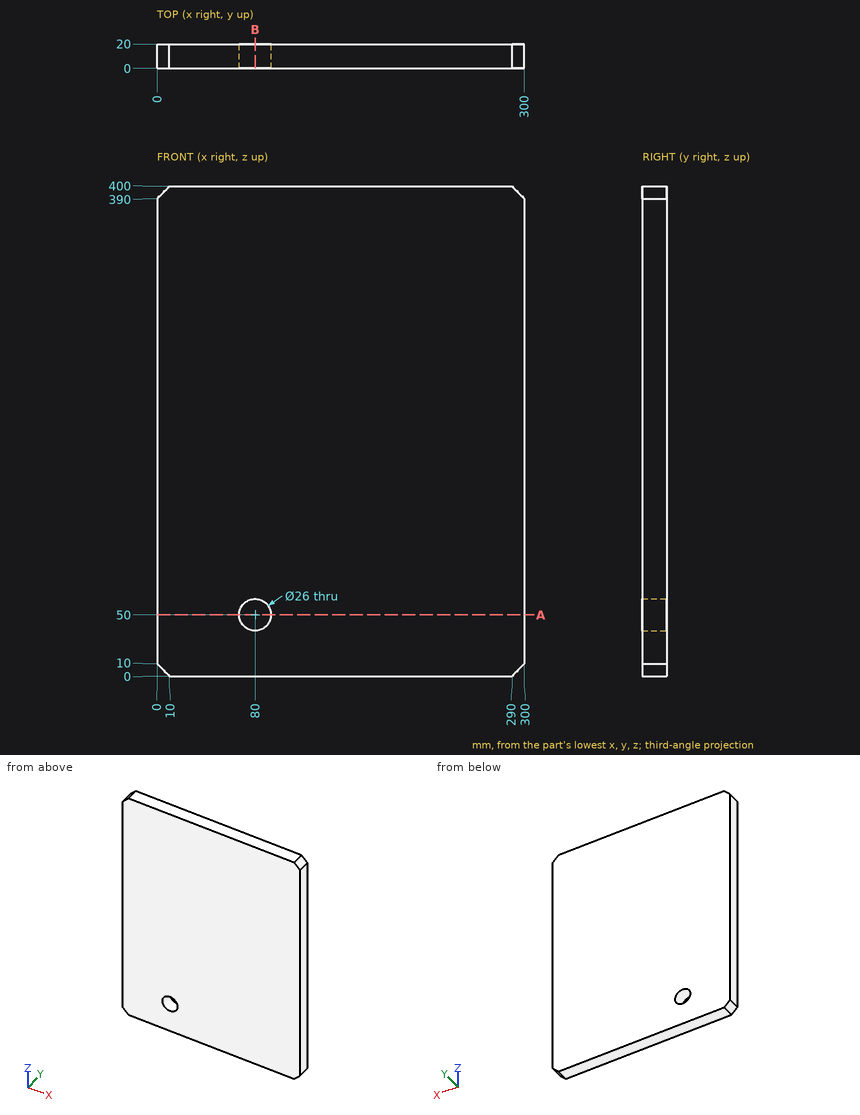
Job drawing, mm, ordinate dimensions from the low corner. One solid piece. Coordinates: 2 decimals unless noted, no trailing zeros. Order: outer loops, then holes, each group sorted by start corner. A loop starts at its lowest first (then second) coordinate and runs counter-clockwise, first axis right, second up. Notation, with made-up numbers: M -5,60.25 L 46,60.25 A19 ccw 46,97.25 Z; hole C 60,88.5 d5. An arc over 180 degrees is marked long. Return JSON: item names as keys, results as strings.
1. Saw through at A-A (z = 50). Give the cut face in (x, y), and give its area (3 significant figures).
Ans:
{"outline": "M 0,0 L 67,0 L 67,20 L 0,20 Z; M 93,0 L 300,0 L 300,20 L 93,20 Z", "area": "5,480 mm^2"}
2. Drill centre lines: probe 1 along Z at (x, y) = (80, 9); probe 2 along X at (y, z) = (8, 50); probe 3 along Z at (x, y) = (77.5, 7). Where is each one in solid material? Low to high.
Ans:
{"probe 1": "0 to 37, 63 to 400", "probe 2": "0 to 67, 93 to 300", "probe 3": "0 to 37.24, 62.76 to 400"}
3. Saw through at B-B (x = 80). Give the cut face in (y, z), and give its area (3 significant figures).
Ans:
{"outline": "M 0,0 L 20,0 L 20,37 L 0,37 Z; M 0,63 L 20,63 L 20,400 L 0,400 Z", "area": "7,480 mm^2"}
4. Flat gauge pin, fed straight in: pin 1 (23.5 mm diameter, centred on x = 80, z = 50, fed in from +Y). Where does the tip first touch, or does it go through?
Ans:
{"pin 1": "through"}
